from build123d import *

# Parameters (mm, degrees)
SKETCH1_R             = 12.5
BOSS_EXTRUDE1_DEPTH   = 26
SKETCH2_R             = 19
BOSS_EXTRUDE2_DEPTH   = 5
BOSS_EXTRUDE3_START   = 2
SKETCH3_R             = 12.5
BOSS_EXTRUDE3_DEPTH   = 2
CHAMFER1_SIZE         = 0.5
SKETCH4_W             = 56.768050843
SKETCH4_H             = 11.338169824
SKETCH4_W_2           = 56.148312297
SKETCH4_H_2           = 14.587502032
CUT_EXTRUDE1_DEPTH    = 38.389838192
SKETCH5_R             = 9.5
CUT_EXTRUDE2_DEPTH    = 41.401113846
M3_TAPPED_HOLE1_D     = 2.5
M3_TAPPED_HOLE1_DEPTH = 7.5
M3_TAPPED_HOLE1_TIP   = 0.751075774
CUT_EXTRUDE3_DEPTH    = 10
SKETCH11_W            = 60.135329508
SKETCH11_H            = 29.448988524
CUT_EXTRUDE4_DEPTH    = 25


with BuildPart() as part:
    # Sketch1 → Boss-Extrude1 (new body)
    with BuildSketch(Plane.XY):
        with Locations(Location((0, 0, 0), (0, 0, 180))):
            Circle(SKETCH1_R)
    extrude(amount=BOSS_EXTRUDE1_DEPTH)

    # Sketch2 → Boss-Extrude2 (add)
    with BuildSketch(Plane(origin=(0, 0, 0), x_dir=(-1, 0, 0), z_dir=(0, 0, -1))):
        Circle(SKETCH2_R)
    extrude(amount=BOSS_EXTRUDE2_DEPTH)

    # Sketch3 → Boss-Extrude3 (add)
    with BuildSketch(Plane(origin=(0, 0, -5), x_dir=(-1, 0, 0), z_dir=(0, 0, -1)).offset(BOSS_EXTRUDE3_START)):
        Circle(SKETCH3_R)
    extrude(amount=-BOSS_EXTRUDE3_DEPTH)

    # Chamfer1
    chamfer1_edges = [part.edges().sort_by_distance(p)[0] for p in [
        (12.5, 0, -7),
        (12.5, 0, 26),
        (19, 0, 0),
        (19, 0, -5),
    ]]
    chamfer(chamfer1_edges, length=CHAMFER1_SIZE)

    # Sketch4 → Cut-Extrude1 (cut, through all)
    with BuildSketch(Plane.XY):
        with Locations((-0.433816982, -19.169084912)):
            Rectangle(SKETCH4_W, SKETCH4_H)
        with Locations((-0.743686256, 20.793751016)):
            Rectangle(SKETCH4_W_2, SKETCH4_H_2)
    extrude(amount=-CUT_EXTRUDE1_DEPTH, mode=Mode.SUBTRACT)

    # Sketch5 → Cut-Extrude2 (cut, through all)
    with BuildSketch(Plane.XY.offset(26)):
        Circle(SKETCH5_R)
    extrude(amount=-CUT_EXTRUDE2_DEPTH, mode=Mode.SUBTRACT)

    # M3 Tapped Hole1
    with Locations(Plane.XY):
        with Locations((16, 0), (-16, 0)):
            Hole(M3_TAPPED_HOLE1_D / 2, depth=M3_TAPPED_HOLE1_DEPTH)
            with Locations((0, 0, -(M3_TAPPED_HOLE1_DEPTH + M3_TAPPED_HOLE1_TIP / 2))):  # 118° drill point
                Cone(0, M3_TAPPED_HOLE1_D / 2, M3_TAPPED_HOLE1_TIP, mode=Mode.SUBTRACT)

    # Sketch10 → Cut-Extrude3 (cut)
    with BuildSketch(Plane.XY):
        Polygon((20.899032633, 6.052740037), (8, 13.5), (20.899032633, 13.5), align=None)
    cut_extrude3 = extrude(amount=-CUT_EXTRUDE3_DEPTH, mode=Mode.SUBTRACT)

    # Mirror1: Cut-Extrude3 across plane
    add(cut_extrude3.mirror(Plane.ZX), mode=Mode.SUBTRACT)

    # Sketch11 → Cut-Extrude4 (cut)
    with BuildSketch(Plane.XY.offset(26)):
        with Locations((5.227667093, -26.724494262)):
            Rectangle(SKETCH11_W, SKETCH11_H)
    extrude(amount=-CUT_EXTRUDE4_DEPTH, mode=Mode.SUBTRACT)


solid = part.part
CAD build for the part. Positions are in the model's coordinates, mm. A direction names the side the tool comes from. Coordinates: 2 decimals unless noted, no trailing zeros. Loops run counter-clockwise (first coordinate to the right, second up) from the corner with the lowest first, then second, coordinate; pieces in that order, holes last. Notation, with made-up numbers: (-18, 33) -> (-14, 33) arc R22 cw to (-14, 45) -> close; hole circle Ø1 at (68.5, 54). An arc over 180 degrees is marked (long way). One line per item, written item: value.
1. Drill centre lines: line 1 (Y direction, x = 0, z = 13.5); line 2 (Y direction, x = -6.5, z = 12); line 3 (X direction, y = -1, z = 17). Where is each one in solid material? Low to high. Write a range as [from, to].
Answers:
line 1: y = [-12, -9.5], [9.5, 12.5]
line 2: y = [-10.68, -6.93], [6.93, 10.68]
line 3: x = [-12.46, -9.45], [9.45, 12.46]
2. Flat gauge pins, fed straight in: P1, Ø8, axis at y = 6.5, z = 16, coming from the +X side; P2, Ø4, axis at x = -3.5, z = 21.5, coming from the -Y side; P3, Ø4, axis at x = 16, y = 0, coming from the -Z side; P4, Ø6, axis at x = 0.5, y = -4, coming from the -Z side (1 decimal). Where does each tip first touch, or does it go through?
Answers:
P1: stops at x = 12.25
P2: stops at y = -12
P3: stops at z = -5
P4: passes through
3. Slice it at B-B on x = 13. Write the cut outline in (y, z).
Answers:
outline: (-10.61, -5) -> (10.61, -5) -> (10.61, 0) -> (-10.61, 0) -> close
4. Which spindle directions (+Z, -Z, +X, -X, +Y, -Y) get a long thin tool onto all of the face, cutting with end or side? Do faces 1 (the face through (2.71, 12.203, 12.572)), 2 (the face through (-11.923, 3.755, -5.76)), 3 (the face through (0, -12, 14)). Say none if no direction does.
Answers:
face 1: +Z
face 2: -Z
face 3: +Z, +X, -X, -Y
5. Slice it at A-A on z = 12. Write the cut outline in (x, y).
Answers:
outline: (-3.5, -12) -> (3.5, -12) arc R12.5 ccw (long way) to start; hole circle Ø19 at (0, 0)
6. Pull direction Y, two halves, no side cores. Call faces 4 (the face through (-18.634, -0.213, -4.865)), 5 (the face through (17.25, 0.05, -2.54)), 6 (the face through (12.626, -10.829, -2.465)), 7 (the face through (13, 0, -5)): pulls with the +Y half, pulls with the -Y half, needs draft (parallel to the pull), parting line crosses it, or undercut.
Answers:
face 4: parting line crosses it
face 5: undercut
face 6: pulls with the -Y half
face 7: needs draft
